Design review of the part built by this model. Coordinates are the model's own, in mm. A direction names the side the tool comes from. Round coordinates to 2 decimals unless told otherwise and drop trailing zeros. Loops run counter-clockwise (first coordinate to the right, second up) from the corner with the lowest first, then second, coordinate; pieces in that order, holes last. Notation, with made-up numbers: (73.25, 49) - (100.25, 49) arc R25 ccw to (100.25, 76) - close; hole circle Ø11 at (21.5, -24). An arc over 180 degrees is marked (long way). Answer as CSV lines item,"result". Start each with the question number.
(1) For P1, Ø4, axis at x = 7, y = -55, coming from the +Z side; P2, Ø1.5, axis at y = -7.5, z = 6.5, coming from the -X side; P3, Ø5, axis at x = 57.5, z = -0.5, coming from the +Y side, all flat-tipped, find the tip position at first contact; note any pin that passes through.
(2) Wall thickness on L1, parallel to X at y = -14, z = -10.25; L2, parallel to X at y = -11, z = -12.5; L3, parallel to X at y = -58, z = -10.5: over which ranges is each line inside the solid? List them lowest first.
(3) Consider section B-B (y = -59). Give the boundary of the cut face in (x, z).
(4) For faces 4 (the flat face through (-35.87, -89.14, 0.21)), 5 (the cylindrical face through (72.9, -65.08, -12.54)), 6 (the cylindrical face through (73, -33, 13)), list the 3-axis set-ups (+Z, -Z, +X, -X, +Y, -Y) from which the entire face can be reached by the end or side of a thin tool; tool diameter is ignored.
(5) Consider section D-D (z = 8). Give the boundary of the cut face in (x, y).
(6) Consider section A-A (x = 0). Give the boundary of the cut face in (y, z).
(7) Consider section C-C (y = -82.5). Count the separate pieces of the cut face and the enclosed holes in it, and give its area (3 significant figures).
(8) Mouldability with a two-part tool opening along X and no side actions: class faces 1 (the cylindrical face through (47.02, -84.9, -12.54)), 2 (the cylindrical face through (-77.05, -30.03, 0.21)), 3 (the flat face through (0, -24, -15)) as released by +X, released by -X, zero draft, split by the parting line, or undercut.
from build123d import *

# Parameters (mm, degrees)
BRACKET_PLATE_DEPTH          = 15
FRONT_FACE_POCKET_DEPTH      = 5
MOUNTING_HOLES_X3_DEPTH      = 129.953479984
MOUNTING_HOLES_X3_DEPTH_BACK = 129.953479984
MOUNTING_HOLES_SKETCH_R      = 10


with BuildPart() as part:
    # Bracket Outline Sketch → Bracket Plate (new, symmetric)
    with BuildSketch(Plane.XY):
        with BuildLine():
            Line((-80, -88), (-80, -40.481444811))
            ThreePointArc((-80, -40.481444811), (-76.967037057, -29.892787979), (-68.78803465, -22.515631526))
            Line((-68.78803465, -22.515631526), (-4.394017325, 8.982906643))
            ThreePointArc((-4.394017325, 8.982906643), (0, 10), (4.394017325, 8.982906643))
            Line((4.394017325, 8.982906643), (68.78803465, -22.515631526))
            ThreePointArc((68.78803465, -22.515631526), (76.967037057, -29.892787979), (80, -40.481444811))
            Line((80, -40.481444811), (80, -88))
            ThreePointArc((80, -88), (76.079830561, -95.939500006), (67.39286793, -97.654162955))
            Line((67.39286793, -97.654162955), (5.21426414, -80.862667644))
            ThreePointArc((5.21426414, -80.862667644), (0, -80.170993555), (-5.21426414, -80.862667644))
            Line((-5.21426414, -80.862667644), (-67.39286793, -97.654162955))
            ThreePointArc((-67.39286793, -97.654162955), (-76.079830561, -95.939500006), (-80, -88))
        make_face()
    extrude(amount=BRACKET_PLATE_DEPTH, both=True)

    # Face Pocket Sketch → Front Face Pocket (cut)
    with BuildSketch(Plane.XY.offset(15)):
        with BuildLine():
            Line((75, -61.007005292), (75, -40.481444811))
            ThreePointArc((75, -40.481444811), (72.725277793, -32.539952187), (66.591025987, -27.007084847))
            Line((66.591025987, -27.007084847), (22.195825808, -5.291031626))
            ThreePointArc((22.195825808, -5.291031626), (17.328625574, -5.555183565), (14.999112859, -9.83686371))
            ThreePointArc((14.999112859, -9.83686371), (0, -25), (-14.999112859, -9.83686371))
            ThreePointArc((-14.999112859, -9.83686371), (-17.328625574, -5.555183565), (-22.195825808, -5.291031626))
            Line((-22.195825808, -5.291031626), (-66.591025987, -27.007084847))
            ThreePointArc((-66.591025987, -27.007084847), (-72.725277793, -32.539952187), (-75, -40.481444811))
            Line((-75, -40.481444811), (-75, -61.007005292))
            ThreePointArc((-75, -61.007005292), (-72.949594192, -65.044318025), (-68.48004236, -65.770378967))
            ThreePointArc((-68.48004236, -65.770378967), (-54.800423598, -68.151249984), (-48.935434642, -80.737052336))
            ThreePointArc((-48.935434642, -80.737052336), (-47.069212384, -84.862736832), (-42.636957008, -85.789651261))
            Line((-42.636957008, -85.789651261), (-6.517830175, -76.035586166))
            ThreePointArc((-6.517830175, -76.035586166), (0, -75.170993555), (6.517830175, -76.035586166))
            Line((6.517830175, -76.035586166), (42.636957008, -85.789651261))
            ThreePointArc((42.636957008, -85.789651261), (47.069212384, -84.862736832), (48.935434642, -80.737052336))
            ThreePointArc((48.935434642, -80.737052336), (54.800423598, -68.151249984), (68.48004236, -65.770378967))
            ThreePointArc((68.48004236, -65.770378967), (72.949594192, -65.044318025), (75, -61.007005292))
        make_face()
    front_face_pocket = extrude(amount=-FRONT_FACE_POCKET_DEPTH, mode=Mode.SUBTRACT)

    # Back Face Pocket Mirror: Front Face Pocket across plane
    add(front_face_pocket.mirror(Plane.XY), mode=Mode.SUBTRACT)

    # Mounting Holes Sketch → Mounting Holes x3 (cut, two sides: drawn at the far end of the back side and taken through both)
    with BuildSketch(Plane.XY.offset(10).offset(-MOUNTING_HOLES_X3_DEPTH_BACK)):
        with Locations((-63.920169439, -80.060499994)):
            Circle(MOUNTING_HOLES_SKETCH_R)
        with Locations((0, -10)):
            Circle(MOUNTING_HOLES_SKETCH_R)
        with Locations((63.920169439, -80.060499994)):
            Circle(MOUNTING_HOLES_SKETCH_R)
    extrude(amount=MOUNTING_HOLES_X3_DEPTH + MOUNTING_HOLES_X3_DEPTH_BACK, mode=Mode.SUBTRACT)


solid = part.part
Determined:
1,P1,"stops at z = 10"
1,P2,"stops at x = -39.62"
1,P3,"stops at y = -15.77"
2,L1,"x = -51.38 to -40, -14.46 to -9.17, 9.17 to 14.46, 40 to 51.38"
2,L2,"x = -45.25 to -33.87, -14.97 to -9.95, 9.95 to 14.97, 33.87 to 45.25"
2,L3,"x = -80 to -75, 75 to 80"
3,outline,"(-80, -15) - (-75, -15) - (-75, -10) - (75, -10) - (75, -15) - (80, -15) - (80, 15) - (75, 15) - (75, 10) - (-75, 10) - (-75, 15) - (-80, 15) - close"
4,face 4,"+Z, -Z, -Y"
4,face 5,"-Z"
4,face 6,"+Z"
5,outline,"(-80, -88) arc R10 ccw to (-67.39, -97.65) - (-5.21, -80.86) arc R20 cw to (5.21, -80.86) - (67.39, -97.65) arc R10 ccw to (80, -88) - (80, -40.48) arc R20 ccw to (68.79, -22.52) - (4.39, 8.98) arc R10 ccw to (-4.39, 8.98) - (-68.79, -22.52) arc R20 ccw to (-80, -40.48) - close; hole circle Ø20 at (-63.92, -80.06); hole circle Ø20 at (0, -10); hole circle Ø20 at (63.92, -80.06)"
6,outline,"(-80.17, -15) - (-75.17, -15) - (-75.17, -10) - (-25, -10) - (-25, -15) - (-20, -15) - (-20, 15) - (-25, 15) - (-25, 10) - (-75.17, 10) - (-75.17, 15) - (-80.17, 15) - close; (0, -15) - (10, -15) - (10, 15) - (0, 15) - close"
7,separate pieces,"4"
7,enclosed holes,"0"
7,area,"2,590 mm^2"
8,face 1,"undercut"
8,face 2,"released by -X"
8,face 3,"zero draft"
